from build123d import *

# Parameters (mm, degrees)
SKETCH_1_W          = 170
SKETCH_1_H          = 60.52
EXTRUDE_1_DEPTH     = 150
SKETCH_2_W          = 150
SKETCH_2_H          = 130
CUT_EXTRUDE_1_DEPTH = 50.52


with BuildPart() as part:
    # 草图1 → 凸台-拉伸1 (new body)
    with BuildSketch(Plane.XY):
        with Locations((-32.516262295, 4.960655738)):
            Rectangle(SKETCH_1_W, SKETCH_1_H)
    extrude(amount=EXTRUDE_1_DEPTH)

    # 草图2 → 切除-拉伸1 (cut)
    with BuildSketch(Plane.XZ.offset(25.299344262)):
        with Locations((-32.516262295, 75)):
            Rectangle(SKETCH_2_W, SKETCH_2_H)
    extrude(amount=-CUT_EXTRUDE_1_DEPTH, mode=Mode.SUBTRACT)


solid = part.part
Here's how the part is built. I have some questions about the finished solid (model axes, mm). A direction names the side the tool comes from. Coordinates: 2 decimals unless noted, no trailing zeros. Write each loop counter-clockwise with the first axis right and the second up, starting at its lowest first coordinate (ties: lowest second). Pieces come first, ordered by that corner, then holes. Notation, with made-up numbers: (25.25, 78) - (77.25, 78) arc R22 ccw to (77.25, 109) - close; hole circle Ø2 at (36.25, 58.25). An arc over 180 degrees is marked (long way). Use one line per item in the form item = value.
1) Suppose I cut it at C-C, the plane y = 0. Write out the boundary of the cut face in (x, z).
Solved:
outline = (-117.52, 0) - (52.48, 0) - (52.48, 150) - (-117.52, 150) - close; hole (-107.52, 10) - (42.48, 10) - (42.48, 140) - (-107.52, 140) - close
2) Thinking about a two-plate mould opening in X: for faces 3 (the flat face through (-34, 35.221, 74)), 4 (the flat face through (-117.516, 5, 74)), 5 (the flat face through (-34, 0, 10)), which applies, released by +X, released by -X, zero draft, split by the parting line, or undercut?
Solved:
face_3 = zero draft
face_4 = released by -X
face_5 = undercut
3) Suppose I cut it at A-A, the plane x = -14. Write out the boundary of the cut face in (y, z).
Solved:
outline = (-25.3, 0) - (35.22, 0) - (35.22, 150) - (-25.3, 150) - (-25.3, 140) - (25.22, 140) - (25.22, 10) - (-25.3, 10) - close
4) Suppose I cut it at B-B, the plane z = 93.5. Write out the boundary of the cut face in (x, y).
Solved:
outline = (-117.52, -25.3) - (-107.52, -25.3) - (-107.52, 25.22) - (42.48, 25.22) - (42.48, -25.3) - (52.48, -25.3) - (52.48, 35.22) - (-117.52, 35.22) - close
5) I'm going to push a flat-ended pin straight in: P1, Ø4, axis at x = -2.5, z = 108.5, coming from the -Y side. Where does the tip first touch, or does it pass through?
Solved:
P1 = 25.22
6) I need wall thicknesses on line 1 (X direction, y = 22, z = 10.5); line 2 (Z direction, x = -6, y = 12.5); line 3 (Y direction, x = 2.5, z = 118). Which ranges of each line are inside material? Lowest first, please.
Solved:
line_1 = -117.52 to -107.52, 42.48 to 52.48
line_2 = 0 to 10, 140 to 150
line_3 = 25.22 to 35.22
7) On a 3-axis mill with a long thin cutter (end or side, diameter ignored), from which of +Z, -Z, +X, -X, +Y, -Y can I reach the whole of each face in a straight line? I mean faces 1 (the flat face through (-34, 0, 140)), 2 (the flat face through (-34, 5, 150)). Say none if no direction works.
Solved:
face_1 = -Y
face_2 = +Z, +X, -X, +Y, -Y
